Part model, mm, in its own coordinate system. A direction names the side the tool comes from. Give positions to 0.01 mm unless a question says otherwise; leave off trailing zeros. Write each loop counter-clockwise with the first axis right and the second up, starting at its lowest first coordinate (ties: lowest second). Pieces come first, ordered by that corner, then holes.
```python
from build123d import *

# Parameters (mm, degrees)
BASE_BLOCK_DEPTH       = 25
CYLINDER_BOSS_SKETCH_R = 25
CYLINDER_BOSS_50_DEPTH = 25
WEB_START              = 10
WEB_BOSS_DEPTH         = 10
BORE_SKETCH_R          = 12.5
BORE_25_DEPTH          = 82.533502
T_SLOT_CUT_DEPTH       = 90.009618
HOLE_SKETCH_R          = 5
HOLE_10_DEPTH          = 77.495661


with BuildPart() as part:
    # Base Profile Sketch → Base Block (new, symmetric)
    with BuildSketch(Plane.XY):
        Polygon((0, 0), (-25, 0), (-62.290509, -21.529686), (-69.265518, -8.25003), (-25, 15), (0, 15), align=None)
    extrude(amount=BASE_BLOCK_DEPTH, both=True)

    # Cylinder Boss Sketch → Cylinder Boss Ø50 (add)
    with BuildSketch(Plane(origin=(0, 0, 0), x_dir=(1, 0, 0), z_dir=(0, 1, 0))):
        with Locations(Location((12.5, 0, 0), (0, 0, 120))):
            Circle(CYLINDER_BOSS_SKETCH_R)
    extrude(amount=CYLINDER_BOSS_50_DEPTH)

    # Web Boss Sketch → Web Boss (add)
    with BuildSketch(Plane.XZ.offset(WEB_START)):
        with BuildLine():
            ThreePointArc((0, 21.650635), (-12.5, 0), (0, -21.650635))
            ThreePointArc((0, -21.650635), (25, -21.650635), (37.5, 0))
            ThreePointArc((37.5, 0), (25, 21.650635), (0, 21.650635))
        make_face()
    extrude(amount=-WEB_BOSS_DEPTH)

    # Bore Sketch → Bore Ø25 (cut, through all)
    with BuildSketch(Plane.XZ.offset(10)):
        with Locations((12.5, 0)):
            Circle(BORE_SKETCH_R)
    extrude(amount=-BORE_25_DEPTH, mode=Mode.SUBTRACT)

    # T-Slot Sketch → T-Slot Cut (cut, through all)
    with BuildSketch(Plane.XY.offset(25)):
        Polygon((-42.70267, 5.701846), (-51.555777, 1.051838), (-49.055777, -3.278289), (-40.402434, 1.717721), align=None)
    extrude(amount=-T_SLOT_CUT_DEPTH, mode=Mode.SUBTRACT)

    # Hole Sketch → Hole Ø10 (cut, through all)
    with BuildSketch(Plane(origin=(-11.580687, 22.048363, 0), x_dir=(0.8853103641838149, 0.4650006011487738, 0), z_dir=(-0.4650006011487738, 0.8853103641838149, 0))):
        with Locations(Location((-55.155754, 0, 0), (0, 0, 180))):
            Circle(HOLE_SKETCH_R)
    extrude(amount=-HOLE_10_DEPTH, mode=Mode.SUBTRACT)


solid = part.part
```
1) Saw through at D-D, the plane x = -21.5. Write the cut outline in (y, z), then the cut area to 3 significant figures.
Answers follow:
outline: (0, -25) - (15, -25) - (15, 25) - (0, 25) - close
area: 750 mm2
2) Saw through at B-B, the plane x = 12.5. Write the cut outline in (y, z), then the cut area to 3 significant figures.
Answers follow:
outline: (-10, -25) - (25, -25) - (25, -12.5) - (-10, -12.5) - close; (-10, 12.5) - (25, 12.5) - (25, 25) - (-10, 25) - close
area: 875 mm2
3) Saw through at A-A, the plane z = -11. Write the cut outline in (x, y).
Answers follow:
outline: (-69.27, -8.25) - (-62.29, -21.53) - (-25, 0) - (-9.95, 0) - (-9.95, -10) - (6.56, -10) - (6.56, 25) - (-9.95, 25) - (-9.95, 15) - (-25, 15) - (-42.7, 5.7) - (-40.4, 1.72) - (-49.06, -3.28) - (-51.56, 1.05) - close; (18.44, -10) - (34.95, -10) - (34.95, 25) - (18.44, 25) - close
4) 3-axis set-ups, long thin cutter, end or side, ignore diameter. For faces 5 (the face through (-50.323, -1.083, 0.35)), 6 (the face through (-44.79, -0.815, 0.35)), 7 (the face through (-15, 0, 0)): which of +Z, -Z, +X, -X, +Y, -Y reach the whole face in a straight line?
Answers follow:
face 5: +Z, -Z, +Y
face 6: +Z, -Z
face 7: -Y
5) Wall check: L1, parallel to Z at x = 12, y = 3 (3 decimals); L2, parallel to Y at x = 23.5, z = 10; L3, parallel to X at y = 11, z = -0.5 (3 decimals). Give the ranges that are in metal, low to high.
Answers follow:
L1: z = -24.995 to -12.49, 12.49 to 24.995
L2: y = -10 to 25
L3: x = -32.616 to 0.01, 24.99 to 37.495
6) Two-plate mould, pull along Z, no slides. Class faces 1 (the face through (-34, 1, -25)), 2 (the face through (0.012, 7.255, 0.55)), 3 (the face through (13, 25, 13)), 4 (the face through (-34, 1, 25)): +Z half, -Z half, draft (parallel to the pull), parting line (faces both ways), or undercut.
Answers follow:
face 1: -Z half
face 2: undercut
face 3: draft
face 4: +Z half
7) Saw through at C-C, the plane y = 18.5. Write the cut outline in (x, z).
Answers follow:
outline: circle Ø50 at (12.5, 0); hole circle Ø25 at (12.5, 0)
8) Pin check, flat tips, straight feed: pin 1 Ø20 at (x, z) = (-17.5, -7) entering from -Y; pin 2 Ø1 at (y, z) = (8, 23) entering from +X; pin 3 Ø12 at (x, z) = (-49.5, 12) entering from -Y. Stop position of each tip, or through.
Answers follow:
pin 1: stops at y = -10
pin 2: stops at x = 23.4
pin 3: stops at y = -17.61
